Verification items for the finished model (mm, model axes). Face numbers are marked on the shaded views. A direction names the side the tool comes from. Give positions to 0.01 mm unless a question says otherwise; leave off trailing zeros. Loops run counter-clockwise (first coordinate to the right, second up) from the corner with the lowest first, then second, coordinate; pieces in that order, holes last. Notation, with made-up numbers: M 58.5,-34.5 L 66.5,-34.5 A17 ccw 66.5,-3.5 Z; hole C 16,33 d5. An arc over 180 degrees is marked long. Use a Markdown table: item, result.
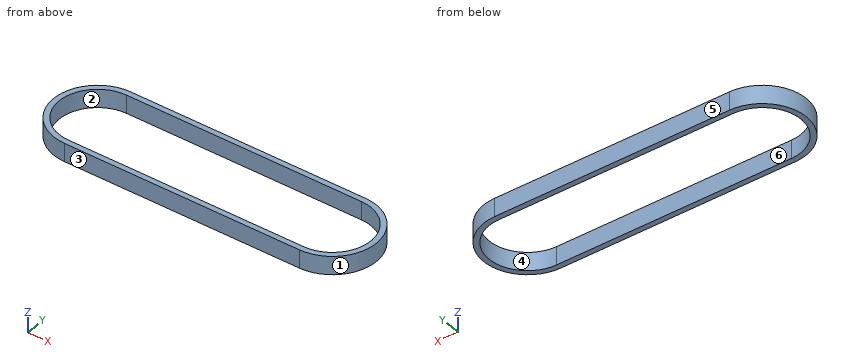
from build123d import *

# Parameters (mm, degrees)
BOSS_EXTRUDE1_DEPTH = 10
SHELL1_T            = -3


with BuildPart() as part:
    # Sketch2 → Boss-Extrude1 (new body)
    with BuildSketch(Plane.XY):
        with BuildLine():
            Line((0, 24), (-130, 24))
            ThreePointArc((-130, 24), (-154, 0), (-130, -24))
            Line((-130, -24), (0, -24))
            ThreePointArc((0, -24), (24, 0), (0, 24))
        make_face()
    extrude(amount=BOSS_EXTRUDE1_DEPTH)

    # Shell1
    shell1_openings = [part.faces().sort_by_distance(p)[0] for p in [
        (-65, 0, 10),
        (-65, 0, 0),
    ]]
    offset(amount=SHELL1_T, openings=shell1_openings, kind=Kind.INTERSECTION)


solid = part.part
(1) Cross-section at B-B on x = -7. Record the cut outline in (y, z), then the cut area to 3 significant figures.
Results below:
| item | result |
|---|---|
| outline | M -24,0 L -21,0 L -21,10 L -24,10 Z; M 21,0 L 24,0 L 24,10 L 21,10 Z |
| area | 60.0 mm^2 |
(2) Set-up check for the marked faces 5 and 6: record each of +Z, -Z, +X, -X, +Y, -Y from which the full face is reachable in a straight line by a thin tool's end or side.
Results below:
| item | result |
|---|---|
| face 5 | +Z, -Z, +X, -X, +Y |
| face 6 | +Z, -Z |
(3) Cross-section at A-A on y = 0. Record the cut outline in (x, z).
Results below:
| item | result |
|---|---|
| outline | M -154,0 L -151,0 L -151,10 L -154,10 Z; M 21,0 L 24,0 L 24,10 L 21,10 Z |
(4) Material ranges on line 1 (X direction, y = -0.5, z = 7.25); line 2 (Y direction, x = -29, z = 5); line 3 (Y direction, x = 5, z = 7), recorded low to high.
Results below:
| item | result |
|---|---|
| line 1 | -153.99 to -150.99, 20.99 to 23.99 |
| line 2 | -24 to -21, 21 to 24 |
| line 3 | -23.47 to -20.4, 20.4 to 23.47 |
(5) Gauge pin test, flat ends, axial feed: P1, Ø6, axis at y = 18.5, z = 1.5, coming from the -X side; P2, Ø5, axis at y = 4.5, z = 1.5, coming from the +X side; P3, Ø2, axis at y = -19, z = 2.5, coming from the -X side. Record the tip position at first contact, or that the pin passes through.
Results below:
| item | result |
|---|---|
| P1 | x = -148.32 |
| P2 | x = 23.92 |
| P3 | x = -145.87 |
(6) Draft check along X on the marked faces 1, 2, 3 and 4. Enter one of: +X half, -X half, draft (parallel to the pull), parting line (faces both ways), or undercut.
Results below:
| item | result |
|---|---|
| face 1 | +X half |
| face 2 | undercut |
| face 3 | draft |
| face 4 | undercut |
(7) Cross-section at C-C on z = 4.5. Record the cut outline in (x, y), then the cut area to 3 significant figures.
Results below:
| item | result |
|---|---|
| outline | M -130,-24 L 0,-24 A24 ccw 0,24 L -130,24 A24 ccw Z; hole M -130,-21 L 0,-21 A21 ccw 0,21 L -130,21 A21 ccw Z |
| area | 1,200 mm^2 |
